Answer from the drawing. Dimensions are ordinates in mm from the lowest x, y and z of the part. A direction names the side the tool comes from. Give positions to 0.01 mm unless a question says otherwise; leave off trailing zeros. Write each loop counter-clockwise with the first axis right and the second up, starting at its lowest first coordinate (ties: lowest second). Pieces come first, ordered by that corner, then holes. Notation, with made-up numbers: M -38,-23 L -14,-23 A13 cw -14,-17 Z; hole C 29,-27 d4. An arc over 180 degrees is marked long. Answer as a JSON object with one key per item and string values.
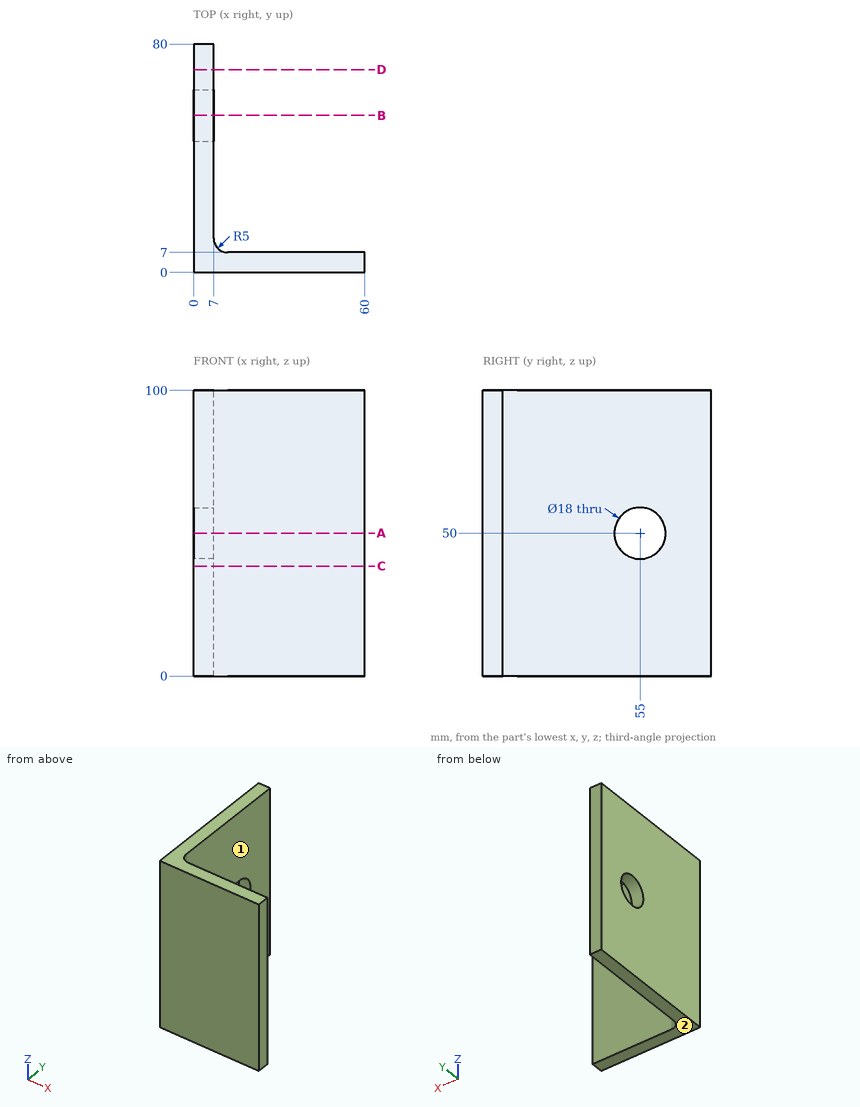
1. For the marked faces 1 and 2, determine the directions among +Z, -Z, +X, -X, +Y, -Y from which every point of the face is accessible in a straight line to the end or side of a thin tool.
Verdict:
{"face 1": "+Z, -Z, +X, +Y", "face 2": "-Z, +X, -X, +Y, -Y"}
2. Flat-ended cylindrical pins translate along their axes: pin 1 (1 mm diameter, centred on x = 37, z = 15, fed in from +Y); pin 2 (12 mm diameter, centred on y = 34, z = 37, fed in from +X). Find the tip coordinate at first contact, or state that the pin passes through.
Verdict:
{"pin 1": "stops at y = 7", "pin 2": "stops at x = 7"}
3. A cutting plane is placed at B-B, the plane y = 55. Give the vertices of the cut face in (x, z).
Verdict:
{"outline": "M 0,0 L 7,0 L 7,41 L 0,41 Z; M 0,59 L 7,59 L 7,100 L 0,100 Z"}
4. A cutting plane is placed at D-D, the plane y = 71. Give the vertices of the cut face in (x, z), plus the area to 3 significant figures.
Verdict:
{"outline": "M 0,0 L 7,0 L 7,100 L 0,100 Z", "area": "700 mm2"}
5. A cutting plane is placed at A-A, the plane z = 50. Give the vertices of the cut face in (x, y).
Verdict:
{"outline": "M 0,0 L 60,0 L 60,7 L 12,7 A5 cw 7,12 L 7,46 L 0,46 Z; M 0,64 L 7,64 L 7,80 L 0,80 Z"}
6. A cutting plane is placed at C-C, the plane z = 38.5. Give the vertices of the cut face in (x, y), plus the area to 3 significant figures.
Verdict:
{"outline": "M 0,0 L 60,0 L 60,7 L 12,7 A5 cw 7,12 L 7,80 L 0,80 Z", "area": "936 mm2"}
7. Consider line 1 along Y through (x, z) = (2.75, 50); line 2 along Y through (x, z) = (23.5, 95.5). Determine where each line is inside the solid, lowest interval first.
Verdict:
{"line 1": "y = 0 to 46, 64 to 80", "line 2": "y = 0 to 7"}
